```python
from build123d import *

# Parameters (mm, degrees)
SKETCH1_R           = 5
BOSS_EXTRUDE1_DEPTH = 3


with BuildPart() as part:
    # Sketch1 → Boss-Extrude1 (new, symmetric)
    with BuildSketch(Plane.XY):
        with BuildLine():
            Line((0, 10), (105, 10))
            ThreePointArc((105, 10), (115, 0), (105, -10))
            Line((105, -10), (0, -10))
            ThreePointArc((0, -10), (-10, 0), (0, 10))
        make_face()
        Circle(SKETCH1_R, mode=Mode.SUBTRACT)
        with Locations((105, 0)):
            Circle(SKETCH1_R, mode=Mode.SUBTRACT)
    extrude(amount=BOSS_EXTRUDE1_DEPTH, both=True)


solid = part.part
```
Can you work these out from the model? Positions are in its coordinate system, mm. Give positions to 0.01 mm unless a question says otherwise; leave off trailing zeros. Write each loop counter-clockwise with the first axis right and the second up, starting at its lowest first coordinate (ties: lowest second). Pieces come first, ordered by that corner, then holes. Notation, with made-up numbers: (56, -13.5) -> (70, -13.5) arc R36 ccw to (70, 23.5) -> close; hole circle Ø10 at (66, 85). An arc over 180 degrees is marked (long way). Write item = value, one per line.
(1) I'm going to push flat-ended pins straight in: P1, Ø2, axis at y = 7, z = 1, coming from the -X side; P2, Ø6, axis at x = 0, y = 0, coming from the -Z side; P3, Ø1, axis at y = -2, z = 2, coming from the +X side. Where does each tip first touch, or does it pass through?
Worked out:
P1 = -8
P2 = through
P3 = 114.89
(2) Suppose I cut it at A-A on y = 0. Write out the boundary of the cut face in (x, z).
Worked out:
outline = (-10, -3) -> (-5, -3) -> (-5, 3) -> (-10, 3) -> close; (5, -3) -> (100, -3) -> (100, 3) -> (5, 3) -> close; (110, -3) -> (115, -3) -> (115, 3) -> (110, 3) -> close
(3) Suppose I cut it at C-C on y = -8. Write out the boundary of the cut face in (x, z), then the cut area to 3 significant figures.
Worked out:
outline = (-6, -3) -> (111, -3) -> (111, 3) -> (-6, 3) -> close
area = 702 mm^2
(4) Thinking about a two-plate mould opening in Y: for faces 1 (the face through (53, 0, -3)), 2 (the face through (109.619, -1.915, -0.042)), 3 (the face through (-1.08, -4.88, -0.04)), 4 (the face through (-10, 0, 0)), which applies, released by +Y, released by -Y, zero draft, split by the parting line, or undercut?
Worked out:
face_1 = zero draft
face_2 = undercut
face_3 = undercut
face_4 = split by the parting line
(5) I need wall thicknesses on probe 1 along Y at (x, z) = (0, -1); probe 2 along X at (y, z) = (-0.75, 0); probe 3 along X at (y, z) = (1, 0.95). Which ranges of each line are inside material? Lowest first, please. Write a range as from..to.
Worked out:
probe_1 = -10..-5, 5..10
probe_2 = -9.97..-4.94, 4.94..100.06, 109.94..114.97
probe_3 = -9.95..-4.9, 4.9..100.1, 109.9..114.95
(6) Suppose I cut it at B-B on z = -0.75. Write out the boundary of the cut face in (x, y).
Worked out:
outline = (0, -10) -> (105, -10) arc R10 ccw to (105, 10) -> (0, 10) arc R10 ccw to start; hole circle Ø10 at (0, 0); hole circle Ø10 at (105, 0)
